Design review of the part shown in the three views and the two pictorial views. Dimensions are in mm from the part's minimum x, y and z. A direction names the side the tool comes from. Coordinates: 2 decimals unless noted, no trailing zeros. Write each loop counter-clockwise with the first axis right and the second up, starting at its lowest first coordinate (ties: lowest second). Pieces come first, ordered by that corner, then holes.
Q1. For pin 1 Ø1.5 at (x, z) = (8, 5) entering from -Y; pin 2 Ø0.8 at (y, z) = (18.5, 5.5) entering from -X; pin 3 Ø1.2 at (x, y) = (17, 19.5) entering from +Z; pin 4 Ø0.8 at (x, y) = (17, 20.5) entering from -Z, all flat-tipped, find the tip position at first contact; note any pin that passes through.
Q2. Take a section at C-C, the plane z = 8.25. Write out the cut boundary in (x, y), plus the area to 3 significant figures.
Q3. Take a section at D-D, the plane y = 5.75. Write out the cut boundary in (x, z).
Q4. For L1, parallel to Z at x = 8, y = 1.2; L2, parallel to X at y = 1.85, z = 5; L3, parallel to Y at x = 8.75, z = 3, list the stretches that pass through material, from the lowest coordinate up.
Q5. For the marked faces 5 and 6, list the 3-axis set-ups (+Z, -Z, +X, -X, +Y, -Y) from which the entire face can be reached by the end or side of a thin tool; tool diameter is ignored.
Q6. Take a section at A-A, the plane z = 5. Write out the cut boundary in (x, y).
Q7. The part is to be moulded in two halves that separate along X. For the marked faces 1, 2, 3 and 4, say which applies: released by +X, released by -X, zero draft, split by the parting line, or undercut.
Q8. Take a section at B-B, the plane x = 8. Write out the cut boundary in (y, z), plus the area to 4 significant figures.
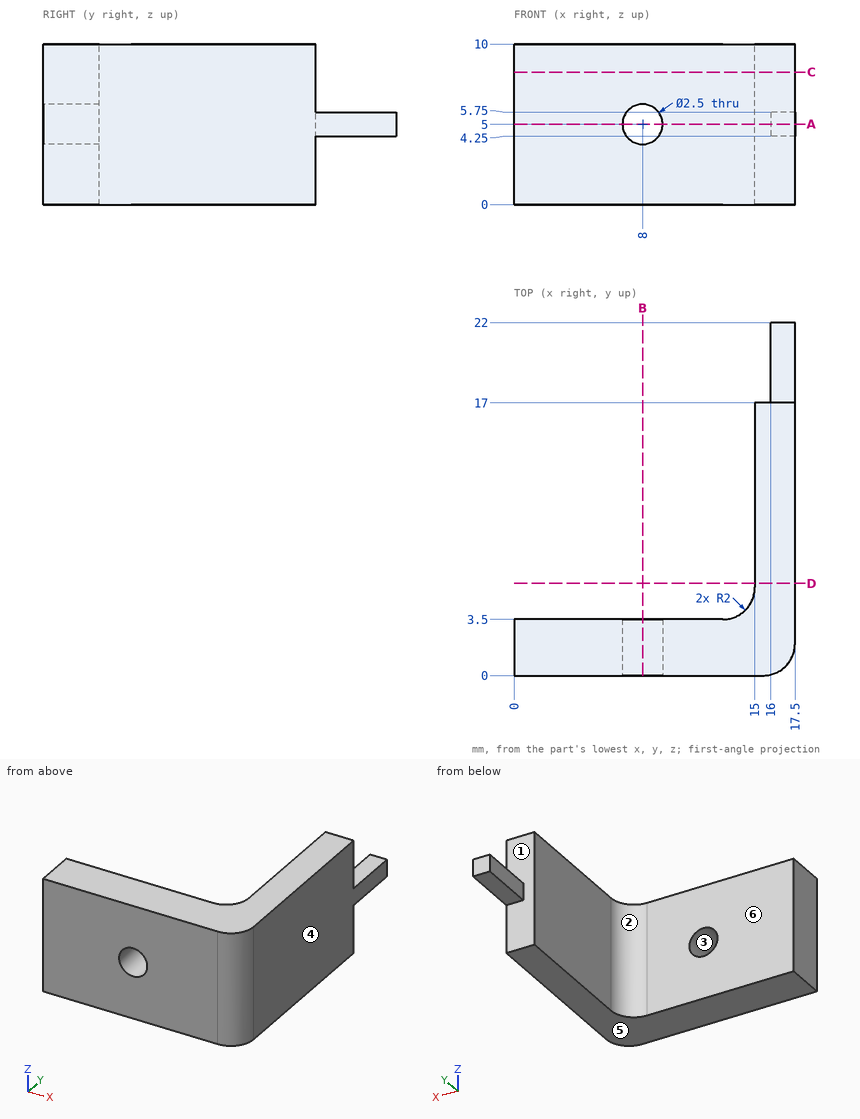
Responses:
1. pin 1: passes through
1. pin 2: stops at x = 16
1. pin 3: stops at z = 5.75
1. pin 4: stops at z = 4.25
2. outline: (0, 0) - (15.5, 0) arc R2 ccw to (17.5, 2) - (17.5, 17) - (15, 17) - (15, 5.5) arc R2 cw to (13, 3.5) - (0, 3.5) - close
2. area: 95.0 mm2
3. outline: (15, 0) - (17.5, 0) - (17.5, 10) - (15, 10) - close
4. L1: z = 0 to 3.75, 6.25 to 10
4. L2: x = 0 to 6.75, 9.25 to 17.49
4. L3: y = 0 to 3.5
5. face 5: -Z, +X, -X, +Y, -Y
5. face 6: +Z, -Z, -X, +Y
6. outline: (0, 0) - (6.75, 0) - (6.75, 3.5) - (0, 3.5) - close; (9.25, 0) - (15.5, 0) arc R2 ccw to (17.5, 2) - (17.5, 22) - (16, 22) - (16, 17) - (15, 17) - (15, 5.5) arc R2 cw to (13, 3.5) - (9.25, 3.5) - close
7. face 1: zero draft
7. face 2: released by -X
7. face 3: undercut
7. face 4: released by +X
8. outline: (0, 0) - (3.5, 0) - (3.5, 3.75) - (0, 3.75) - close; (0, 6.25) - (3.5, 6.25) - (3.5, 10) - (0, 10) - close
8. area: 26.25 mm2
